Answer from the drawing. Dimensions are ordinates in mm from the lowest x, y and z of the part. A direction names the side the tool comes from. Give positions to 0.01 mm unless a question says otherwise; leave off trailing zeros. Loops run counter-clockwise (first coordinate to the right, second up) from the corner with the lowest first, then second, coordinate; pieces in that order, holes last.
(1) Find section B-B, the plane x = 20. Write down the section's boundary in (y, z).
(2) Find section D-D, the plane z = 20. Write down the section's boundary in (x, y).
(3) Which of the six approach directions +Z, -Z, +X, -X, +Y, -Y give full straight-line access (tool end or side, diameter ignored) to the marked faces 4 and 5?
(4) Find section C-C, the plane y = 2.75. Write down the section's boundary in (x, z), then the cut area to 3 significant figures.
(5) Determine the mould class of the marked faces 1, 2 and 3 for opening direction X: pulls with the +X half, pulls with the -X half, needs draft (parallel to the pull), parting line crosses it, or undercut.
(6) Find section A-A, the plane z = 4. Write down the section's boundary in (x, y), then the cut area to 3 significant figures.
(7) This flat-tipped pin is pushed along its axis until it touches: P1, Ø8, axis at x = 9, y = 10.5, coming from the +Z side. Where does it stop, or does it pass through?
(8) Straight lines are drawn through the part: probe 1 along Z at (x, y) = (36, 1.15); probe 2 along Y at (x, z) = (25.5, 5.25); probe 3 along Z at (x, y) = (4, 12). For each, find the intervals that lie inside material, in ascending order.
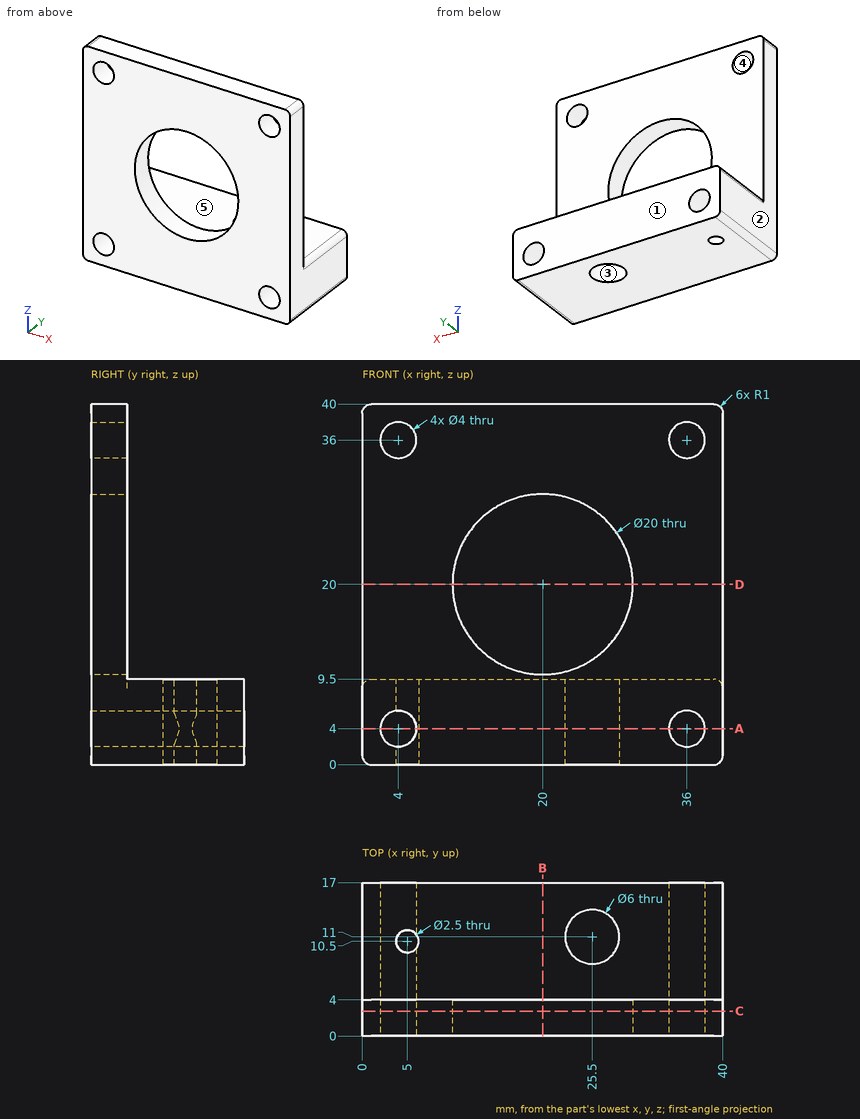
Entries:
1. outline: (0, 0) - (17, 0) - (17, 9.5) - (4, 9.5) - (4, 10) - (0, 10) - close; (0, 30) - (4, 30) - (4, 40) - (0, 40) - close
2. outline: (0, 0) - (10, 0) - (10, 4) - (0, 4) - close; (30, 0) - (40, 0) - (40, 4) - (30, 4) - close
3. face 4: +Y, -Y
3. face 5: +Z, +X, -X, +Y
4. outline: (0, 1) arc R1 ccw to (1, 0) - (39, 0) arc R1 ccw to (40, 1) - (40, 39) arc R1 ccw to (39, 40) - (1, 40) arc R1 ccw to (0, 39) - close; hole circle Ø4 at (4, 4); hole circle Ø4 at (4, 36); hole circle Ø20 at (20, 20); hole circle Ø4 at (36, 4); hole circle Ø4 at (36, 36)
4. area: 1,230 mm2
5. face 1: needs draft
5. face 2: pulls with the -X half
5. face 3: undercut
6. outline: (0, 0) - (2, 0) - (2, 17) - (0, 17) - close; (6, 0) - (34, 0) - (34, 17) - (6, 17) - (6, 11.25) arc R1.25 cw to (6, 9.75) - close; (38, 0) - (40, 0) - (40, 17) - (38, 17) - close; hole circle Ø6 at (25.5, 11)
6. area: 515 mm2
7. P1: stops at z = 9.5
8. probe 1: z = 0 to 2, 6 to 34, 38 to 40
8. probe 2: y = 0 to 8, 14 to 17
8. probe 3: z = 0 to 2, 6 to 9.5
